Work out the finished part from the listing and answer in its coordinate system (mm). A direction names the side the tool comes from. Give positions to 0.01 mm unless a question says otherwise; leave off trailing zeros. Order: outer loops, then holes, each group sorted by start corner. A loop starts at its lowest first (then second) coordinate and runs counter-clockwise, first axis right, second up. Notation, with made-up numbers: (-36, 21) - (-3, 21) arc R13 ccw to (-3, 25) - close; hole circle Ø4 at (71, -26.5). An arc over 180 degrees is marked (long way). Put each result on its own line as item: value.
```python
from build123d import *

# Parameters (mm, degrees)
SKETCH_1_W          = 115
SKETCH_1_H          = 53
EXTRUDE_1_DEPTH     = 53
SKETCH_2_W          = 46
SKETCH_2_H          = 28
CUT_EXTRUDE_1_DEPTH = 83.568153667
SKETCH_3_R          = 2.75
CUT_EXTRUDE_2_DEPTH = 83.568153667


with BuildPart() as part:
    # 草图1 → 凸台-拉伸1 (new body)
    with BuildSketch(Plane(origin=(0, 0, 0), x_dir=(1, 0, 0), z_dir=(0, 1, 0))):
        Rectangle(SKETCH_1_W, SKETCH_1_H)
    extrude(amount=EXTRUDE_1_DEPTH)

    # 草图2 → 切除-拉伸1 (cut, through all)
    with BuildSketch(Plane(origin=(0, 53, 0), x_dir=(1, 0, 0), z_dir=(0, 1, 0))):
        with Locations((-57.5, -26.5)):
            Rectangle(SKETCH_2_W, SKETCH_2_H)
        with Locations((-57.5, 26.5)):
            Rectangle(SKETCH_2_W, SKETCH_2_H)
    extrude(amount=-CUT_EXTRUDE_1_DEPTH, mode=Mode.SUBTRACT)

    # 草图3 → 切除-拉伸2 (cut, through all)
    with BuildSketch(Plane(origin=(0, 53, 0), x_dir=(1, 0, 0), z_dir=(0, 1, 0))):
        with Locations(Location((-28.5, 19, 0), (0, 0, 270))):
            Circle(SKETCH_3_R)
        with Locations(Location((51.5, 19, 0), (0, 0, 270))):
            Circle(SKETCH_3_R)
        with Locations(Location((51.5, -19, 0), (0, 0, 270))):
            Circle(SKETCH_3_R)
        with Locations(Location((-28.5, -19, 0), (0, 0, 270))):
            Circle(SKETCH_3_R)
    extrude(amount=-CUT_EXTRUDE_2_DEPTH, mode=Mode.SUBTRACT)


solid = part.part
```
(1) Section B-B, the plane x = 51.5 is taken. Write down the section's boundary in (y, z).
Geometry check:
outline: (0, -26.5) - (53, -26.5) - (53, -21.75) - (0, -21.75) - close; (0, -16.25) - (53, -16.25) - (53, 16.25) - (0, 16.25) - close; (0, 21.75) - (53, 21.75) - (53, 26.5) - (0, 26.5) - close
(2) Section D-D, the plane x = -48 is taken. Write down the section's boundary in (y, z), then the cut area to 4 significant figures.
Geometry check:
outline: (0, -12.5) - (53, -12.5) - (53, 12.5) - (0, 12.5) - close
area: 1,325 mm²
(3) A tool of negligible diameter and unlimited length cuts with its end or side. For faces 1 (the face through (11, 26, 26.5)), 2 (the face through (-46, 27, 12.5)), from which of +Z, -Z, +X, -X, +Y, -Y can it reach the whole face along a straight path? Write none if from no direction.
Geometry check:
face 1: +Z, +X, -X, +Y, -Y
face 2: +Z, -X, +Y, -Y
(4) Given pin 1 (11.5 mm diameter, centred on x = -47, y = 21, fed in from -Z); pin 2 (5 mm diameter, centred on x = 51.5, z = 19, fed in from -Y); pin 3 (7 mm diameter, centred on y = 33.5, z = -22.5, fed in from -X), each flat-ended and moving along its own axis, determine where each tip first touches the part or whether it passes through.
Geometry check:
pin 1: stops at z = -12.5
pin 2: passes through
pin 3: stops at x = -34.5
(5) Section A-A, the plane z = -19 is taken. Write down the section's boundary in (x, y).
Geometry check:
outline: (-34.5, 0) - (-31.25, 0) - (-31.25, 53) - (-34.5, 53) - close; (-25.75, 0) - (48.75, 0) - (48.75, 53) - (-25.75, 53) - close; (54.25, 0) - (57.5, 0) - (57.5, 53) - (54.25, 53) - close
(6) Straight lines are drawn through the part: line 1 (X direction, y = 47, z = -19); line 2 (Z direction, x = -27, y = 9.5); line 3 (Z direction, x = 51, y = 23). For each, find the intervals that lie inside material, in ascending order.
Geometry check:
line 1: x = -34.5 to -31.25, -25.75 to 48.75, 54.25 to 57.5
line 2: z = -26.5 to -21.3, -16.7 to 16.7, 21.3 to 26.5
line 3: z = -26.5 to -21.7, -16.3 to 16.3, 21.7 to 26.5
(7) Section C-C, the plane y = 39.5 is taken. Write down the section's boundary in (x, z), then the cut area to 3 significant figures.
Geometry check:
outline: (-57.5, -12.5) - (-34.5, -12.5) - (-34.5, -26.5) - (57.5, -26.5) - (57.5, 26.5) - (-34.5, 26.5) - (-34.5, 12.5) - (-57.5, 12.5) - close; hole circle Ø5.5 at (-28.5, -19); hole circle Ø5.5 at (-28.5, 19); hole circle Ø5.5 at (51.5, -19); hole circle Ø5.5 at (51.5, 19)
area: 5,360 mm²
(8) Determine the mould class of faces 3 (the face through (-25.773, 26.871, 18.642)), 4 (the face through (-34.5, 27, -19)), 5 (the face through (-46, 27, -12.5)) for opening direction X: pulls with the +X half, pulls with the -X half, needs draft (parallel to the pull), parting line crosses it, or undercut.
Geometry check:
face 3: undercut
face 4: pulls with the -X half
face 5: needs draft
